Read the model definition and answer for the solid it produces. Units are mm, in the model's axes. A direction names the side the tool comes from. Give positions to 0.01 mm unless a question says otherwise; leave off trailing zeros. Order: outer loops, then holes, each group sorted by start corner. A loop starts at its lowest first (then second) coordinate and runs counter-clockwise, first axis right, second up. Notation, with made-up numbers: M 19,41 L 62,41 A24 ccw 62,78 Z; hole C 79.5,49 d11. An arc over 180 degrees is marked long. One line per item, written item: value.
from build123d import *

# Parameters (mm, degrees)
SKETCH_1_R          = 10
EXTRUDE_1_DEPTH     = 20
SKETCH_3_R          = 12.5
EXTRUDE_2_DEPTH     = 12
SKETCH_2_R          = 4.5
CUT_EXTRUDE_1_DEPTH = 27.69269563
CHAMFER_2_SIZE      = 0.5


with BuildPart() as part:
    # 草图1 → 凸台-拉伸1 (new body)
    with BuildSketch(Plane(origin=(0, 0, 0), x_dir=(1, 0, 0), z_dir=(0, 1, 0))):
        with Locations(Location((0, 0, 0), (0, 0, 270))):
            Circle(SKETCH_1_R)
    extrude(amount=EXTRUDE_1_DEPTH)

    # 草图3 → 凸台-拉伸2 (add)
    with BuildSketch(Plane(origin=(0, 0, 0), x_dir=(-1, 0, 0), z_dir=(0, -1, 0))):
        with Locations(Location((0, 0, 0), (0, 0, 90))):
            Circle(SKETCH_3_R)
    extrude(amount=-EXTRUDE_2_DEPTH)

    # 草图2 → 切除-拉伸1 (cut, through all)
    with BuildSketch(Plane(origin=(0, 20, 0), x_dir=(1, 0, 0), z_dir=(0, 1, 0))):
        with Locations(Location((0, 0, 0), (0, 0, 270))):
            Circle(SKETCH_2_R)
    extrude(amount=-CUT_EXTRUDE_1_DEPTH, mode=Mode.SUBTRACT)

    # 倒角2
    chamfer_2_edges = [part.edges().sort_by_distance(p)[0] for p in [
        (0, 20, -10),
        (0, 12, 12.5),
        (0, 0, 12.5),
    ]]
    chamfer(chamfer_2_edges, length=CHAMFER_2_SIZE)


solid = part.part
1) Each of these flat-tipped pins is pushed along its axis until it touches: pin 1 Ø8 at (x, y) = (7.5, 17.5) entering from -Z; pin 2 Ø2 at (y, z) = (14.5, -7.5) entering from +X. Where does it stop, or does it pass through?
Reported:
pin 1: stops at z = -9.37
pin 2: stops at x = 7.6
2) Determine the mould class of faces 1 (the face through (3.755, 5.923, -11.923)), 2 (the face through (1.352, 10.14, 4.292)), 3 (the face through (2.2, 20, 4.1)) for opening direction Z: +Z half, -Z half, draft (parallel to the pull), parting line (faces both ways), or undercut.
Reported:
face 1: parting line
face 2: undercut
face 3: draft
3) Find section D-D, the plane y = 16.5. Write down the section's boundary in (x, z).
Reported:
outline: C 0,0 d20; hole C 0,0 d9
4) Consider probe 1 along X at (y, z) = (13, 0); probe 2 along Y at (x, z) = (-9.5, -3.25); probe 3 along X at (y, z) = (4.75, 0). Determine where each line is inside the solid, lowest interval first.
Reported:
probe 1: x = -10 to -4.5, 4.5 to 10
probe 2: y = 0 to 12
probe 3: x = -12.5 to -4.5, 4.5 to 12.5
5) Which of the six approach directions +Z, -Z, +X, -X, +Y, -Y give full straight-line access (tool end or side, diameter ignored) to faces 4 (the face through (0, 0, -5)), 5 (the face through (9, 12, 5))?
Reported:
face 4: +Z, -Z, +X, -X, -Y
face 5: +Y
6) Find section C-C, the plane y = 6.5. Write down the section's boundary in (x, z), plus the area to 3 significant figures.
Reported:
outline: C 0,0 d25; hole C 0,0 d9
area: 427 mm^2
7) Find section A-A, the plane x = 0. Write down the section's boundary in (y, z), plus the area to 3 significant figures.
Reported:
outline: M 0,-12 L 0.5,-12.5 L 11.5,-12.5 L 12,-12 L 12,-10 L 19.5,-10 L 20,-9.5 L 20,-4.5 L 0,-4.5 Z; M 0,4.5 L 20,4.5 L 20,9.5 L 19.5,10 L 12,10 L 12,12 L 11.5,12.5 L 0.5,12.5 L 0,12 Z
area: 279 mm^2
8) Find section B-B, the plane z = 0. Write down the section's boundary in (x, y), plus the area to 3 significant figures.
Reported:
outline: M -12.5,0.5 L -12,0 L -4.5,0 L -4.5,20 L -9.5,20 L -10,19.5 L -10,12 L -12,12 L -12.5,11.5 Z; M 4.5,0 L 12,0 L 12.5,0.5 L 12.5,11.5 L 12,12 L 10,12 L 10,19.5 L 9.5,20 L 4.5,20 Z
area: 279 mm^2
